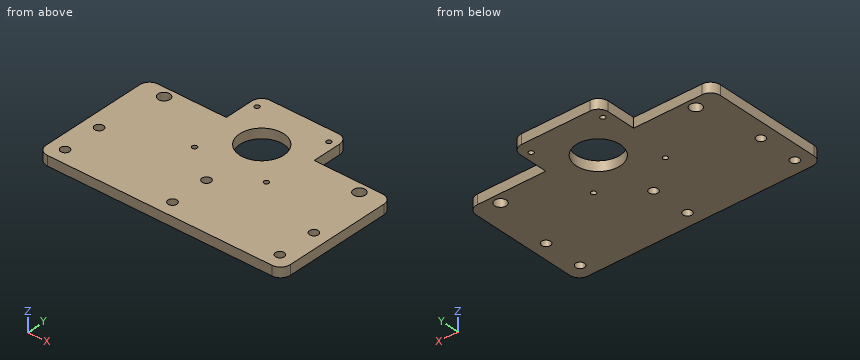
```python
from build123d import *

# Parameters (mm, degrees)
SKETCH_1_W                = 250
SKETCH_1_H                = 170
EXTRUDE_1_DEPTH           = 5
SKETCH_2_W                = 80
SKETCH_2_H                = 40
CUT_EXTRUDE_1_DEPTH       = 10
HOLE_WIZARD_9_0_9_1_D     = 9
PATTERN_LINEAR_1_COUNT    = 3
PATTERN_LINEAR_1_PITCH    = 110
HOLE_WIZARD_12_0_12_1_D   = 12
SKETCH_7_R                = 22.5
CUT_EXTRUDE_2_DEPTH       = 10
HOLE_WIZARD_M6_1_D        = 5
PATTERN_LINEAR_3_COUNT    = 2
PATTERN_LINEAR_3_PITCH    = 73.54
PATTERN_LINEAR_4_COUNT    = 2
PATTERN_LINEAR_4_PITCH    = 73.54
PATTERN_LINEAR_4_COPY_1_D = 5
FILLET_1_R                = 10


with BuildPart() as part:
    # 草图1 → 凸台-拉伸1 (new, symmetric)
    with BuildSketch(Plane.XY):
        Rectangle(SKETCH_1_W, SKETCH_1_H)
    extrude(amount=EXTRUDE_1_DEPTH, both=True)

    # 草图2 → 切除-拉伸1 (cut)
    with BuildSketch(Plane.XY.offset(5)):
        with Locations((85, 65)):
            Rectangle(SKETCH_2_W, SKETCH_2_H)
    cut_extrude_1 = extrude(amount=-CUT_EXTRUDE_1_DEPTH, mode=Mode.SUBTRACT)

    # 镜向1: 切除-拉伸1 across plane
    add(cut_extrude_1.mirror(Plane(origin=(0, 0, 0), x_dir=(0, 0, 1), z_dir=(1, 0, 0))), mode=Mode.SUBTRACT)

    # Ø9.0 (9) 直径孔1 (through all)
    with Locations(Plane.XY.offset(5)):
        with Locations((-110, -70), (-110, -30)):
            hole_wizard_9_0_9_1 = Hole(HOLE_WIZARD_9_0_9_1_D / 2)

    # 阵列(线性)1: Ø9.0 (9) 直径孔1 ×3
    with Locations(*[(i * PATTERN_LINEAR_1_PITCH, 0, 0) for i in range(1, PATTERN_LINEAR_1_COUNT)]):
        add(hole_wizard_9_0_9_1, mode=Mode.SUBTRACT)

    # Ø12.0 (12) 直径孔1 (through all)
    with Locations(Plane.XY.offset(5)):
        with Locations((-100, 35), (100, 35)):
            Hole(HOLE_WIZARD_12_0_12_1_D / 2)

    # 草图7 → 切除-拉伸2 (cut)
    with BuildSketch(Plane.XY.offset(5)):
        with Locations((0, 35)):
            Circle(SKETCH_7_R)
    extrude(amount=-CUT_EXTRUDE_2_DEPTH, mode=Mode.SUBTRACT)

    # M6 螺纹孔1 (through all)
    with Locations(Plane.XY.offset(5)):
        with Locations((-36.77, 71.77)):
            hole_wizard_m6_1 = Hole(HOLE_WIZARD_M6_1_D / 2)

    # 阵列(线性)3: M6 螺纹孔1 ×2
    with Locations(*[(0, -i * PATTERN_LINEAR_3_PITCH, 0) for i in range(1, PATTERN_LINEAR_3_COUNT)]):
        add(hole_wizard_m6_1, mode=Mode.SUBTRACT)

    # 阵列(线性)4: M6 螺纹孔1 ×2
    with Locations(*[(i * PATTERN_LINEAR_4_PITCH, 0, 0) for i in range(1, PATTERN_LINEAR_4_COUNT)]):
        add(hole_wizard_m6_1, mode=Mode.SUBTRACT)

    # 阵列(线性)4 copy 1 (through all)
    with Locations(Plane(origin=(73.54, -73.54, 5), x_dir=(1, 0, 0), z_dir=(0, 0, 1))):
        with Locations((-36.77, 71.77)):
            Hole(PATTERN_LINEAR_4_COPY_1_D / 2)

    # 圆角1
    fillet_1_edges = [part.edges().sort_by_distance(p)[0] for p in [
        (125, 45, 0),
        (45, 85, 0),
        (-125, 45, 0),
        (-45, 85, 0),
        (125, -85, 0),
        (-125, -85, 0),
    ]]
    fillet(fillet_1_edges, radius=FILLET_1_R)


solid = part.part
```
Model file for the job. Use its own axes, mm. Coordinates: 2 decimals unless noted, no trailing zeros. Order: outer loops, then holes, each group sorted by start corner. A loop starts at its lowest first (then second) coordinate and runs counter-clockwise, first axis right, second up. Notation, with made-up numbers: (82, 78) - (103, 78) arc R32 ccw to (103, 111) - close; hole circle Ø4 at (22, 45). An arc over 180 degrees is marked (long way). Return JSON: item names as keys, results as strings. Group by question number.
1) Flat gauge pins, fed straight in: P1, Ø8, axis at x = 0, y = -30, coming from the -Z side; P2, Ø1.5, axis at x = -42, z = 1, coming from the +Y side; P3, Ø5, axis at y = 55.5, z = -0.5, coming from the -X side; P4, Ø3, axis at y = 64.5, z = -1.5, coming from the +X side. Where does each tip first touch, or does it go through?
2) Probe line 1 (X direction, y = -1.77, z = 1); line 2 (Y direction, x = -110, z = -0.75); line 3 (Y direction, x = 0, z = -0.75). List the from-to ranges inside material, lowest first. Write a range as from..to.
3) Saw through at C-C, the plane z = 2. Count the separate pieces of the cut face and the enclosed holes in it, plus the area to 3 significant figures.
4) Saw through at A-A, the plane y = -1.77. Write the cut outline in (x, z).
5) Saw through at B-B, the plane x = 100. Write the cut outline in (y, z).
6) Saw through at D-D, the plane x = 0. Write the cut outline in (y, z), plus the area to 3 significant figures.
Values found:
{
 "1": {"P1": "passes through", "P2": "stops at y = 82.81", "P3": "stops at x = -45", "P4": "stops at x = 45"},
 "2": {"line 1": "x = -125..-39.27, -34.27..34.27, 39.27..125", "line 2": "y = -85..-74.5, -65.5..-34.5, -25.5..45", "line 3": "y = -85..-74.5, -65.5..-34.5, -25.5..12.5, 57.5..85"},
 "3": {"separate pieces": "1", "enclosed holes": "13", "area": "33,700 mm²"},
 "4": {"outline": "(-125, -5) - (-39.27, -5) - (-39.27, 5) - (-125, 5) - close; (-34.27, -5) - (34.27, -5) - (34.27, 5) - (-34.27, 5) - close; (39.27, -5) - (125, -5) - (125, 5) - (39.27, 5) - close"},
 "5": {"outline": "(-85, -5) - (29, -5) - (29, 5) - (-85, 5) - close; (41, -5) - (45, -5) - (45, 5) - (41, 5) - close"},
 "6": {"outline": "(-85, -5) - (-74.5, -5) - (-74.5, 5) - (-85, 5) - close; (-65.5, -5) - (-34.5, -5) - (-34.5, 5) - (-65.5, 5) - close; (-25.5, -5) - (12.5, -5) - (12.5, 5) - (-25.5, 5) - close; (57.5, -5) - (85, -5) - (85, 5) - (57.5, 5) - close", "area": "1,070 mm²"}
}
